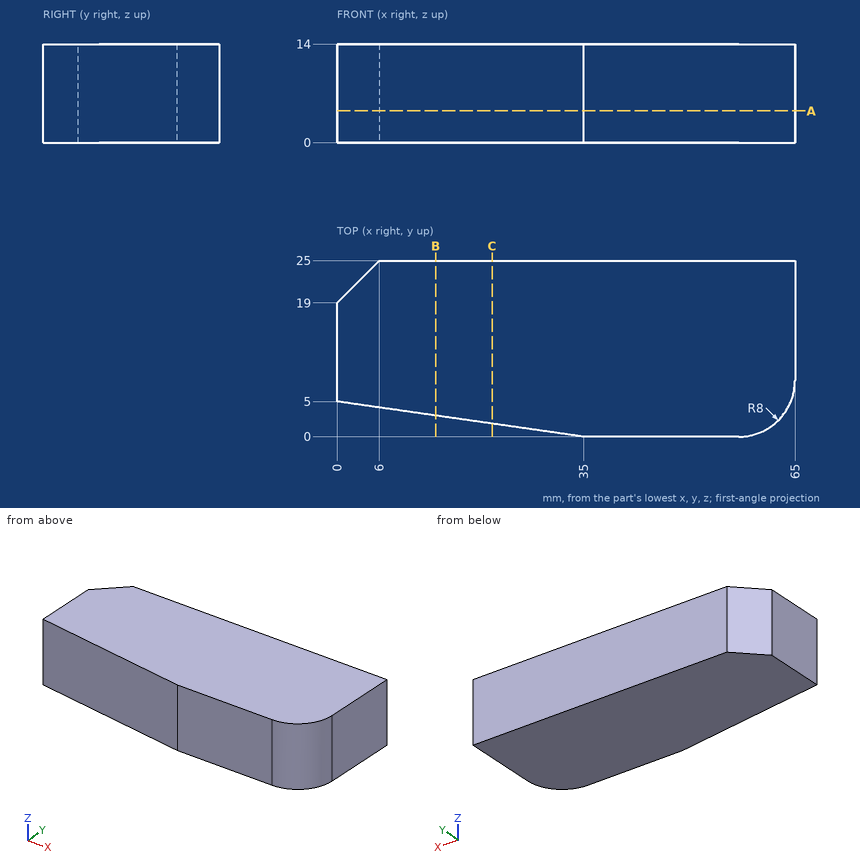
Study the drawing (mm; zero at the part's minimum x, y, z) and answer. Round coordinates to 2 decimals unless told otherwise and drop trailing zeros. Order: outer loops, then holes, each group sorted by start corner. A loop starts at its lowest first (then second) coordinate and runs counter-clockwise, first axis right, second up. Notation, with made-up numbers: (8.5, 50) -> (25.5, 50) arc R8 cw to (25.5, 55) -> close; hole circle Ø3 at (11.5, -27.5). An arc over 180 degrees is marked (long way). Write each question's results on one line, items separated by ' | '. Start each with the question number.
Q1. Find section C-C (x = 22). Determine the outline of the cut face in (y, z).
Q2. Find section A-A (z = 4.5). Determine the outline of the cut face in (x, y).
Q3. Find section B-B (x = 14). Determine the outline of the cut face in (y, z), then the cut area to 3 significant figures.
Q4. Straight lines are drawn through the part: probe 1 along Y at (x, z) = (16, 6.5); probe 2 along Y at (x, z) = (59, 11); probe 3 along X at (y, z) = (7.5, 12.25). For each, find the intervals that lie inside material, in ascending order. Write a range as from..to.
Worked answers:
1) outline: (1.86, 0) -> (25, 0) -> (25, 14) -> (1.86, 14) -> close
2) outline: (0, 5) -> (35, 0) -> (57, 0) arc R8 ccw to (65, 8) -> (65, 25) -> (6, 25) -> (0, 19) -> close
3) outline: (3, 0) -> (25, 0) -> (25, 14) -> (3, 14) -> close | area: 308 mm2
4) probe 1: y = 2.71..25 | probe 2: y = 0.25..25 | probe 3: x = 0..64.98
